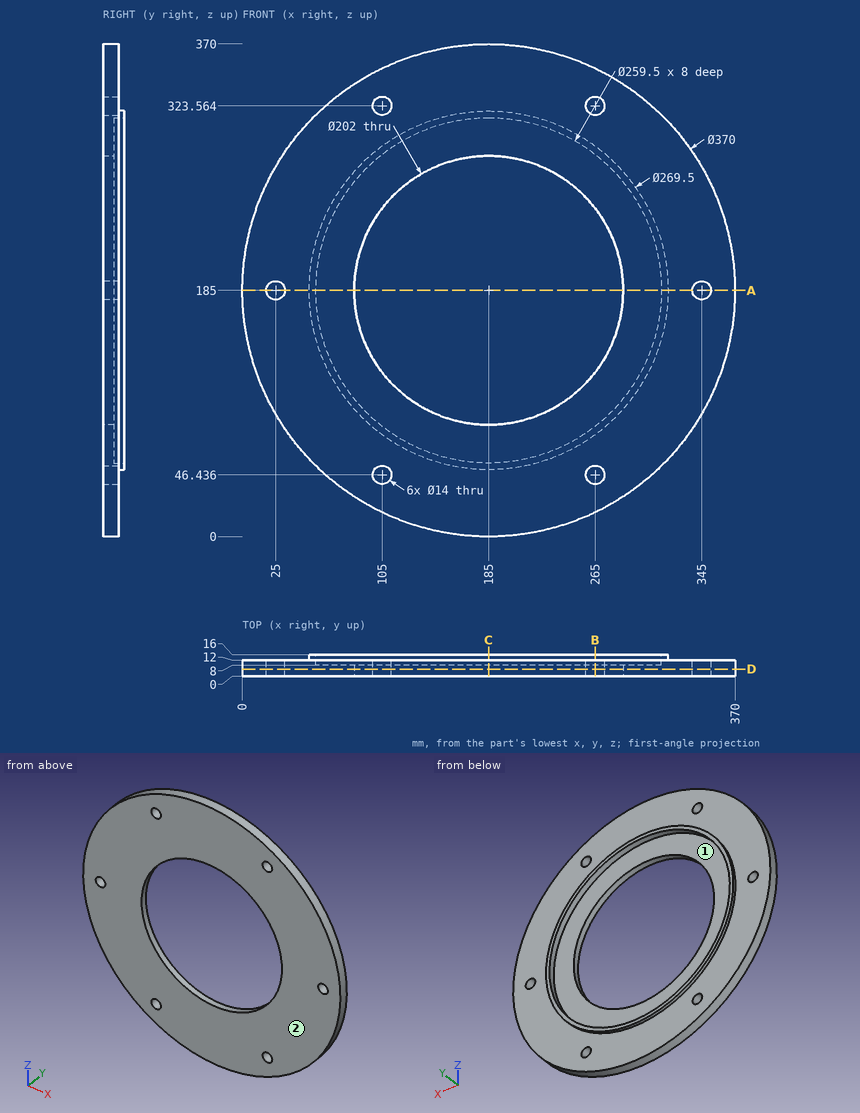
Could you check a few things on this drawing? It's one solid part, dimensions in mm from its lowest x, y, z. Coordinates: 2 decimals unless noted, no trailing zeros. Write each loop counter-clockwise with the first axis right and the second up, starting at its lowest first coordinate (ties: lowest second). Pieces come first, ordered by that corner, then holes.
Q1. Imagine slicing it at C-C, the plane x = 185. List the corners of the cut face in (y, z) for me.
Results found:
outline: (0, 0) - (12, 0) - (12, 50.25) - (16, 50.25) - (16, 55.25) - (8, 55.25) - (8, 84) - (0, 84) - close; (0, 286) - (8, 286) - (8, 314.75) - (16, 314.75) - (16, 319.75) - (12, 319.75) - (12, 370) - (0, 370) - close
Q2. Imagine slicing it at A-A, the plane z = 185. List the corners of the cut face in (x, y) for me.
Results found:
outline: (0, 0) - (18, 0) - (18, 12) - (0, 12) - close; (32, 0) - (84, 0) - (84, 8) - (55.25, 8) - (55.25, 16) - (50.25, 16) - (50.25, 12) - (32, 12) - close; (286, 0) - (338, 0) - (338, 12) - (319.75, 12) - (319.75, 16) - (314.75, 16) - (314.75, 8) - (286, 8) - close; (352, 0) - (370, 0) - (370, 12) - (352, 12) - close
Q3. Please list where these lines run through material, in increasing order: L1, parallel to X at y = 1, z = 181.5; L2, parallel to Z at x = 183, y = 5.5; L3, parallel to Y at x = 49, z = 72.5.
Results found:
L1: x = 0.03 to 18.94, 31.06 to 84.06, 285.94 to 338.94, 351.06 to 369.97
L2: z = 0.01 to 84.02, 285.98 to 369.99
L3: y = 0 to 12
Q4. Imagine slicing it at B-B, the plane x = 265. List the corners of the cut face in (y, z) for me.
Results found:
outline: (0, 18.19) - (12, 18.19) - (12, 39.44) - (0, 39.44) - close; (0, 53.44) - (12, 53.44) - (12, 76.57) - (16, 76.57) - (16, 82.85) - (8, 82.85) - (8, 123.35) - (0, 123.35) - close; (0, 246.65) - (8, 246.65) - (8, 287.15) - (16, 287.15) - (16, 293.43) - (12, 293.43) - (12, 316.56) - (0, 316.56) - close; (0, 330.56) - (12, 330.56) - (12, 351.81) - (0, 351.81) - close
Q5. Imagine slicing it at D-D, the plane y = 5.25. List the corners of the cut face in (x, z) for me.
Results found:
outline: circle Ø370 at (185, 185); hole circle Ø14 at (25, 185); hole circle Ø202 at (185, 185); hole circle Ø14 at (105, 46.44); hole circle Ø14 at (105, 323.56); hole circle Ø14 at (265, 46.44); hole circle Ø14 at (265, 323.56); hole circle Ø14 at (345, 185)
Q6. For P1, Ø8, axis at x = 61.5, z = 262, coming from the -Y side; P2, Ø1.5, axis at y = 13.5, z = 130.5, coming from the +X side; P3, Ø1.5, axis at y = 3, z = 74.5, coming from the -X side; P4, Ø4, axis at y = 3.5, z = 162, coming from the -X side, each with a flat end and sliding along its axis, tell me the tip position at first contact or that it passes through.
Results found:
P1: stops at y = 0
P2: stops at x = 308.57
P3: stops at x = 36.07
P4: stops at x = 1.2
Q7. If we mould it in two halves opening along X, with no side actions, what happens to the marked faces 1 and 2? For each: +X half, -X half, draft (parallel to the pull), parting line (faces both ways), or undercut.
Results found:
face 1: undercut
face 2: draft
